```python
from build123d import *

# Parameters (mm, degrees)
HUB_BASE_25_SKETCH_R       = 12.5
HUB_BASE_25_DEPTH          = 10
HUB_SECTION_1_50_SKETCH_R  = 25
HUB_SECTION_1_50_DEPTH     = 10
HUB_NECK_1_25_SKETCH_R     = 12.5
HUB_NECK_1_25_DEPTH        = 15
HUB_SECTION_2_50_SKETCH_R  = 25
HUB_SECTION_2_50_DEPTH     = 15
HUB_NECK_2_25_SKETCH_R     = 12.5
HUB_NECK_2_25_DEPTH        = 10
HUB_TOP_50_SKETCH_R        = 25
HUB_TOP_50_DEPTH           = 10
ARM_BLOCK_SKETCH_W         = 25
ARM_BLOCK_SKETCH_H         = 15
ARM_BLOCK_DEPTH            = 25
ARM_WEB_PROFILE_SKETCH_W   = 50
ARM_WEB_PROFILE_SKETCH_H   = 25
ARM_WEB_PROFILE_SKETCH_W_2 = 50.02861625
ARM_WEB_DEPTH              = 25
ARM_START                  = -10
ARM_NOTCH_CUT_DEPTH        = 10
NOTCH_FILLER_SKETCH_R      = 25
NOTCH_FILLER_BOSS_DEPTH    = 10
HUB_BORE_25_DEPTH          = 34
HUB_BORE_25_DEPTH_BACK     = 80
HUB_BORE_25_SKETCH_R       = 12.5
DOVETAIL_RAIL_DEPTH        = 50
RAIL_GROOVE_CUT_DEPTH      = 271
RAIL_GROOVE_CUT_DEPTH_BACK = 142
RAIL_HOLE_10_DEPTH         = 179
RAIL_HOLE_10_DEPTH_BACK    = 179
RAIL_HOLE_10_SKETCH_R      = 5


with BuildPart() as part:
    # Hub Base _25 Sketch → Hub Base _25 (new body)
    with BuildSketch(Plane(origin=(0, 0, 0), x_dir=(1, 0, 0), z_dir=(0, 1, 0))):
        with Locations(Location((0, 0, 0), (0, 0, 270))):
            Circle(HUB_BASE_25_SKETCH_R)
    extrude(amount=HUB_BASE_25_DEPTH)

    # Hub Section 1 _50 Sketch → Hub Section 1 _50 (add)
    with BuildSketch(Plane(origin=(0, 10, 0), x_dir=(1, 0, 0), z_dir=(0, 1, 0))):
        with Locations(Location((0, 0, 0), (0, 0, 270))):
            Circle(HUB_SECTION_1_50_SKETCH_R)
    extrude(amount=-HUB_SECTION_1_50_DEPTH)

    # Hub Neck 1 _25 Sketch → Hub Neck 1 _25 (add)
    with BuildSketch(Plane(origin=(0, 10, 0), x_dir=(1, 0, 0), z_dir=(0, 1, 0))):
        with Locations(Location((0, 0, 0), (0, 0, 270))):
            Circle(HUB_NECK_1_25_SKETCH_R)
    extrude(amount=HUB_NECK_1_25_DEPTH)

    # Hub Section 2 _50 Sketch → Hub Section 2 _50 (add)
    with BuildSketch(Plane(origin=(0, 25, 0), x_dir=(1, 0, 0), z_dir=(0, 1, 0))):
        with Locations(Location((0, 0, 0), (0, 0, 270))):
            Circle(HUB_SECTION_2_50_SKETCH_R)
    extrude(amount=-HUB_SECTION_2_50_DEPTH)

    # Hub Neck 2 _25 Sketch → Hub Neck 2 _25 (add)
    with BuildSketch(Plane(origin=(0, 25, 0), x_dir=(1, 0, 0), z_dir=(0, 1, 0))):
        with Locations(Location((0, 0, 0), (0, 0, 270))):
            Circle(HUB_NECK_2_25_SKETCH_R)
    extrude(amount=HUB_NECK_2_25_DEPTH)

    # Hub Top _50 Sketch → Hub Top _50 (add)
    with BuildSketch(Plane(origin=(0, 35, 0), x_dir=(1, 0, 0), z_dir=(0, 1, 0))):
        with Locations(Location((0, 0, 0), (0, 0, 270))):
            Circle(HUB_TOP_50_SKETCH_R)
    extrude(amount=-HUB_TOP_50_DEPTH)



with BuildPart() as body_2:
    # Arm Block Sketch → Arm Block (new, symmetric)
    with BuildSketch(Plane.XY):
        with Locations((-37.5, 17.5)):
            Rectangle(ARM_BLOCK_SKETCH_W, ARM_BLOCK_SKETCH_H)
    extrude(amount=ARM_BLOCK_DEPTH, both=True)


with BuildPart() as part_1:
    add(part.part)

    add(body_2.part)  # Arm Web merges body 2
    # Arm Web Profile Sketch → Arm Web (add)
    with BuildSketch(Plane(origin=(0, 0, 0), x_dir=(1, 0, 0), z_dir=(0, 1, 0))):
        with Locations((-25, 12.5)):
            Rectangle(ARM_WEB_PROFILE_SKETCH_W, ARM_WEB_PROFILE_SKETCH_H)
        with Locations((-25.014308125, -12.5)):
            Rectangle(ARM_WEB_PROFILE_SKETCH_W_2, ARM_WEB_PROFILE_SKETCH_H)
    extrude(amount=ARM_WEB_DEPTH)

    # Arm Notch Sketch → Arm Notch Cut (cut)
    with BuildSketch(Plane.XZ.offset(ARM_START)):
        with BuildLine():
            Line((-2.42391296, 25), (-50.02861625, 25))
            Line((-50.02861625, 25), (-50.02861625, 0))
            Line((-50.02861625, 0), (-50, 0))
            Line((-50, 0), (-50, -25))
            Line((-50, -25), (-2.42391296, -25))
            ThreePointArc((-2.42391296, -25), (-25.117232213, 0), (-2.42391296, 25))
        make_face()
        with BuildLine():
            Line((0, 25), (-2.42391296, 25))
            ThreePointArc((-2.42391296, 25), (-25.117232213, 0), (-2.42391296, -25))
            Line((-2.42391296, -25), (0, -25))
            Line((0, -25), (0, 25))
        make_face()
        with BuildLine():
            Line((0, 25), (0, -25))
            ThreePointArc((0, -25), (25, 0), (0, 25))
        make_face()
    extrude(amount=ARM_NOTCH_CUT_DEPTH, mode=Mode.SUBTRACT)

    # Notch Filler Sketch → Notch Filler Boss (add)
    with BuildSketch(Plane.XZ.offset(-10)):
        with Locations(Location((0, 0, 0), (0, 0, 90))):
            Circle(NOTCH_FILLER_SKETCH_R)
    extrude(amount=NOTCH_FILLER_BOSS_DEPTH)

    # Hub Bore _25 Sketch → Hub Bore _25 (cut, two sides: drawn at the far end of the back side and taken through both)
    with BuildSketch(Plane(origin=(0, 35, 0), x_dir=(1, 0, 0), z_dir=(0, 1, 0)).offset(-HUB_BORE_25_DEPTH_BACK)):
        with Locations(Location((0, 0, 0), (0, 0, 90))):
            Circle(HUB_BORE_25_SKETCH_R)
    extrude(amount=HUB_BORE_25_DEPTH + HUB_BORE_25_DEPTH_BACK, mode=Mode.SUBTRACT)

    # Dovetail Rail Sketch → Dovetail Rail (add)
    with BuildSketch(Plane.XY.offset(25)):
        Polygon((-50.02861625, 10), (-86.834695911, -11.25), (-93.329886439, 0), (-50.02861625, 25), align=None)
    extrude(amount=-DOVETAIL_RAIL_DEPTH)

    # Rail Groove Sketch → Rail Groove Cut (cut, two sides: drawn at the far end of the back side and taken through both)
    with BuildSketch(Plane.XY.offset(25).offset(-RAIL_GROOVE_CUT_DEPTH_BACK)):
        Polygon((-80.339505382, 7.5), (-77.839505382, 3.169872981), (-60.518997307, 13.169872981), (-63.018997307, 17.5), align=None)
    extrude(amount=RAIL_GROOVE_CUT_DEPTH + RAIL_GROOVE_CUT_DEPTH_BACK, mode=Mode.SUBTRACT)

    # Rail Hole _10 Sketch → Rail Hole _10 (cut, two sides: drawn at the far end of the back side and taken through both)
    with BuildSketch(Plane(origin=(-23.33247161, 40.413026294, 0), x_dir=(0.8660254037844379, 0.5000000000000013, 0), z_dir=(-0.5000000000000013, 0.8660254037844379, 0)).offset(-RAIL_HOLE_10_DEPTH_BACK)):
        with Locations((-73.326052589, 0)):
            Circle(RAIL_HOLE_10_SKETCH_R)
    extrude(amount=RAIL_HOLE_10_DEPTH + RAIL_HOLE_10_DEPTH_BACK, mode=Mode.SUBTRACT)


solid = part_1.part
```
Build history of the part. All positions in model axes, mm. A direction names the side the tool comes from. Round coordinates to 2 decimals unless told otherwise and drop trailing zeros. Order: outer loops, then holes, each group sorted by start corner. A loop starts at its lowest first (then second) coordinate and runs counter-clockwise, first axis right, second up. Notation, with made-up numbers: (31, 47) - (59, 47) arc R22 ccw to (59, 59) - close; hole circle Ø10 at (68.25, 1.5). An arc over 180 degrees is marked (long way). Use a Markdown table: item, result.
1) Saw through at D-D on y = 30. Write the cut outline in (x, z), and give its area (3 significant figures).
Recorded:
| item | result |
|---|---|
| outline | circle Ø50 at (0, 0); hole circle Ø25 at (0, 0) |
| area | 1,470 mm² |
2) Tool access for faces 4 (the face through (-5.9, 0, -11.5)), 5 (the face through (-79.11, 5.37, -0.35)), 6 (the face through (-61.75, 15.3, -0.35)), 7 (the face through (-68.174, -0.476, 0.35)): list every direction of +Z, -Z, +X, -X, +Y, -Y with a clear straight run to the whole face (end or side of a thin tool).
Recorded:
| item | result |
|---|---|
| face 4 | +Z, -Z, +X, -Y |
| face 5 | +Z, -Z, +Y |
| face 6 | +Z, -Z, -X |
| face 7 | +Z, -Z, -Y |
3) Saw through at B-B on z = -19.5. Write the cut outline in (x, y), and give its area (3 significant figures).
Recorded:
| item | result |
|---|---|
| outline | (-93.33, 0) - (-86.83, -11.25) - (-50.03, 10) - (-50.03, 25) - (-63.02, 17.5) - (-60.52, 13.17) - (-77.84, 3.17) - (-80.34, 7.5) - close; (-50, 10) - (-15.64, 10) - (-15.64, 0) - (15.64, 0) - (15.64, 35) - (-15.64, 35) - (-15.64, 25) - (-50, 25) - close |
| area | 2,110 mm² |
4) Wall check: L1, parallel to X at y = 8.5, z = 0; L2, parallel to X at y = 8, z = 0; L3, parallel to Y at x = -16, z = -6. Give the ranges that are in metal, low to high.
Recorded:
| item | result |
|---|---|
| L1 | x = -68.61 to -52.63, -25 to -12.5, 12.5 to 25 |
| L2 | x = -69.47 to -53.49, -25 to -12.5, 12.5 to 25 |
| L3 | y = 0 to 35 |
5) Flat gauge pins, fed straight in: pin 1 Ø6 at (x, z) = (-48.5, 7) entering from +Y; pin 2 Ø20 at (x, z) = (0, 0) entering from -Y; pin 3 Ø12 at (y, z) = (27.5, -14) entering from -X; pin 4 Ø8 at (y, z) = (11, -7.5) entering from -X. Where does each tip first touch, or does it go through?
Recorded:
| item | result |
|---|---|
| pin 1 | stops at y = 25 |
| pin 2 | passes through |
| pin 3 | stops at x = -56.09 |
| pin 4 | stops at x = -81.21 |
6) Pull direction X, two halves, no side cores. Call faces 1 (the face through (-25, 17, -25)), 2 (the face through (-56.61, 21.2, 0.35)), 3 (the face through (-36, 10, 0)): pulls with the +X half, pulls with the -X half, needs draft (parallel to the pull), parting line crosses it, or undercut.
Recorded:
| item | result |
|---|---|
| face 1 | needs draft |
| face 2 | pulls with the -X half |
| face 3 | undercut |
7) Saw through at C-C on z = 15. Write the cut outline in (x, y), and give its area (3 significant figures).
Recorded:
| item | result |
|---|---|
| outline | (-93.33, 0) - (-86.83, -11.25) - (-50.03, 10) - (-20, 10) - (-20, 0) - (20, 0) - (20, 35) - (-20, 35) - (-20, 25) - (-50.03, 25) - (-63.02, 17.5) - (-60.52, 13.17) - (-77.84, 3.17) - (-80.34, 7.5) - close |
| area | 2,350 mm² |
8) Saw through at A-A on x = -6.5. Write the cut outline in (y, z), and give its area (3 significant figures).
Recorded:
| item | result |
|---|---|
| outline | (0, -24.14) - (10, -24.14) - (10, -25) - (25, -25) - (25, -24.14) - (35, -24.14) - (35, -10.68) - (0, -10.68) - close; (0, 10.68) - (35, 10.68) - (35, 24.14) - (25, 24.14) - (25, 25) - (10, 25) - (10, 24.14) - (0, 24.14) - close |
| area | 968 mm² |
